Part model, mm, in its own coordinate system. Face numbers are marked on the shaded views. A direction names the side the tool comes from. Give positions to 0.01 mm unless a question says otherwise; leave off trailing zeros. Write each loop counter-clockwise with the first axis right and the second up, starting at its lowest first coordinate (ties: lowest second). Pieces come first, ordered by that corner, then holes. Notation, with made-up numbers: M 69,78 L 114,78 A27 cw 114,108 Z; hole C -28,41 d10. An arc over 180 degrees is marked long. Use a Markdown table: item, result.
```python
from build123d import *

# Parameters (mm, degrees)
BASE_PLATE_SKETCH_W    = 76
BASE_PLATE_SKETCH_H    = 60
BASE_PLATE_DEPTH       = 16
UPRIGHT_WALL_DEPTH     = 76
WALL_NOTCH_SKETCH_W    = 76
WALL_NOTCH_SKETCH_H    = 25
WALL_NOTCH_DEPTH       = 16
ARM_BLOCK_SKETCH_W     = 120
ARM_BLOCK_SKETCH_H     = 20
ARM_BLOCK_DEPTH        = 40
ARM_LUG_DEPTH          = 40
ARM_SIDE_CUT_A_DEPTH   = 12
ARM_START              = -12
ARM_SIDE_CUT_B_DEPTH   = 12
PIVOT_HOLE_20_SKETCH_R = 10
PIVOT_HOLE_20_DEPTH    = 16


with BuildPart() as part:
    # Base Plate Sketch → Base Plate (new body)
    with BuildSketch(Plane.XY):
        with Locations((38, 30)):
            Rectangle(BASE_PLATE_SKETCH_W, BASE_PLATE_SKETCH_H)
    extrude(amount=BASE_PLATE_DEPTH)

    # Upright Wall Sketch → Upright Wall (add)
    with BuildSketch(Plane(origin=(76, 0, 0), x_dir=(0, 0, -1), z_dir=(1, 0, 0))):
        Polygon((-16, 60), (-41, 60), (-46, 60), (-46, 35), (-16, 35), align=None)
    extrude(amount=-UPRIGHT_WALL_DEPTH)

    # Wall Notch Sketch → Wall Notch (cut)
    with BuildSketch(Plane.XY.offset(46)):
        with Locations((38, 47.5)):
            Rectangle(WALL_NOTCH_SKETCH_W, WALL_NOTCH_SKETCH_H)
    extrude(amount=-WALL_NOTCH_DEPTH, mode=Mode.SUBTRACT)

    # Arm Block Sketch → Arm Block (add)
    with BuildSketch(Plane.ZY):
        with Locations((90, 50)):
            Rectangle(ARM_BLOCK_SKETCH_W, ARM_BLOCK_SKETCH_H)
    extrude(amount=-ARM_BLOCK_DEPTH)

    # Arm Lug Sketch → Arm Lug (add)
    with BuildSketch(Plane(origin=(40, 0, 0), x_dir=(0, 0, -1), z_dir=(1, 0, 0))):
        with BuildLine():
            Line((-53.649750889, 98.032798162), (-150, 60))
            Line((-150, 60), (-30, 60))
            Line((-30, 60), (-25, 60))
            Line((-25, 60), (-25, 80))
            ThreePointArc((-25, 80), (-33.167646012, 96.124372828), (-50.99953991, 99.078928714))
            Line((-50.99953991, 99.078928714), (-53.649750889, 98.032798162))
        make_face()
    extrude(amount=-ARM_LUG_DEPTH)

    # Arm Side Cut A Sketch → Arm Side Cut A (cut)
    with BuildSketch(Plane(origin=(40, 0, 0), x_dir=(0, 0, -1), z_dir=(1, 0, 0))):
        with BuildLine():
            Line((-53.649750889, 98.032798162), (-150, 60))
            Line((-150, 60), (-30, 60))
            Line((-30, 60), (-25, 60))
            Line((-25, 60), (-25, 80))
            ThreePointArc((-25, 80), (-33.167646012, 96.124372828), (-50.99953991, 99.078928714))
            Line((-50.99953991, 99.078928714), (-53.649750889, 98.032798162))
        make_face()
    extrude(amount=-ARM_SIDE_CUT_A_DEPTH, mode=Mode.SUBTRACT)

    # Arm Side Cut B Sketch → Arm Side Cut B (cut)
    with BuildSketch(Plane.ZY.offset(ARM_START)):
        with BuildLine():
            Line((25, 80), (25, 60))
            Line((25, 60), (150, 60))
            Line((150, 60), (53.649750889, 98.032798162))
            Line((53.649750889, 98.032798162), (50.99953991, 99.078928714))
            ThreePointArc((50.99953991, 99.078928714), (33.167646012, 96.124372828), (25, 80))
        make_face()
    extrude(amount=ARM_SIDE_CUT_B_DEPTH, mode=Mode.SUBTRACT)

    # Pivot Hole Ø20 Sketch → Pivot Hole Ø20 (cut)
    with BuildSketch(Plane(origin=(28, 0, 0), x_dir=(0, 0, -1), z_dir=(1, 0, 0))):
        with Locations((-45, 80)):
            Circle(PIVOT_HOLE_20_SKETCH_R)
    extrude(amount=-PIVOT_HOLE_20_DEPTH, mode=Mode.SUBTRACT)


solid = part.part
```
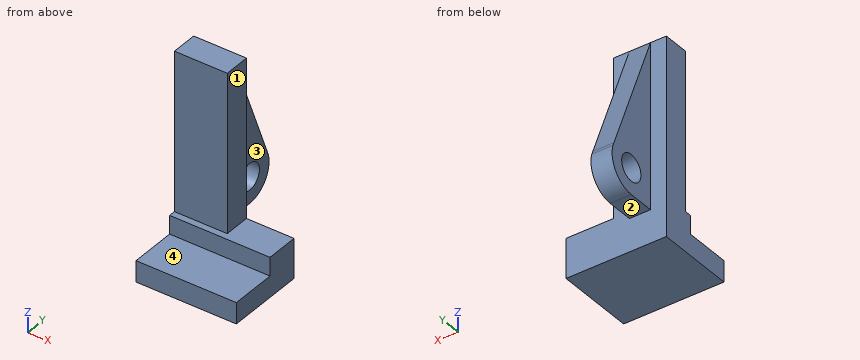
1. Cut at A-A, the plane z = 45. Give the cut face in (x, y), then the cut area to 3 significant figures.
Findings below:
| item | result |
|---|---|
| outline | M 0,40 L 40,40 L 40,60 L 28,60 L 28,70 L 12,70 L 12,60 L 0,60 Z; M 12,90 L 28,90 L 28,100 L 12,100 Z |
| area | 1,120 mm2 |
2. Drop flat-ended pins along their axis: P1, Ø6, axis at y = 53, z = 115, coming from the +X side; P2, Ø12, axis at y = 76.5, z = 113, coming from the -X side; P3, Ø4, axis at x = 49, z = 26.5, coming from the -Y side. Give the stop position or say it passes through.
Findings below:
| item | result |
|---|---|
| P1 | x = 40 |
| P2 | x = 12 |
| P3 | y = 35 |
3. Drill centre lines: L1, parallel to Y at x = 22.75, z = 45; L2, parallel to Z at x = 36.5, y = 19; L3, parallel to Y at x = 11, z = 21.5. Where is each one in solid material? Low to high.
Findings below:
| item | result |
|---|---|
| L1 | 40 to 70, 90 to 100 |
| L2 | 0 to 16 |
| L3 | 35 to 60 |
4. Cut at B-B, the plane x = 35. Give the cut face in (y, z), then the cut area to 3 significant figures.
Findings below:
| item | result |
|---|---|
| outline | M 0,0 L 60,0 L 60,150 L 40,150 L 40,30 L 35,30 L 35,16 L 0,16 Z |
| area | 3,710 mm2 |
5. Cut at D-D, the plane y = 27.5. Give the cut face in (x, z), then the cut area to 3 significant figures.
Findings below:
| item | result |
|---|---|
| outline | M 0,0 L 76,0 L 76,16 L 0,16 Z |
| area | 1,220 mm2 |
6. Tool access for the marked faces 1, 2, 3 and 4: list every direction of +Z, -Z, +X, -X, +Y, -Y with a clear straight run to the whole face (end or side of a thin tool).
Findings below:
| item | result |
|---|---|
| face 1 | +Z, +X, +Y, -Y |
| face 2 | -Z, +X, -X, +Y |
| face 3 | +Z, -Z, +X, +Y |
| face 4 | +Z, +X, -X, -Y |
7. Cut at C-C, the plane z = 108. Give the cut face in (x, y).
Findings below:
| item | result |
|---|---|
| outline | M 0,40 L 40,40 L 40,60 L 28,60 L 28,76.58 L 12,76.58 L 12,60 L 0,60 Z |
